Here's the drawing with two shaded views (mm, measured from the low corner). I have some questions. Coordinates: 2 decimals unless noted, no trailing zeros. Write each loop counter-clockwise with the first axis right and the second up, starting at its lowest first coordinate (ties: lowest second). Pieces come first, ordered by that corner, then holes.
Item 1: If we section it at C-C (x = 171.5): Please give me the cut outline in (y, z).
Item 2: If we section it at B-B (z = 68.5): Please give me the cut outline in (x, y).
Item 3: If I drill on line 1 (X direction, y = 1.9, z = 74); line 2 (Z direction, x = 232, y = 1.25); line 3 (Z direction, x = 141, y = 0.3), over which ranges is the centre line in solid material (lowest first)?
Item 4: I'm going to push flat-ended pins straight in: pin 1 Ø1.5 at (x, y) = (19, 2) entering from +Z; pin 2 Ø1.5 at (y, z) = (2, 161.5) entering from +X; pin 3 Ø1.5 at (y, z) = (2, 161.5) entering from -X. Where does each tip first touch, or does it pass through?
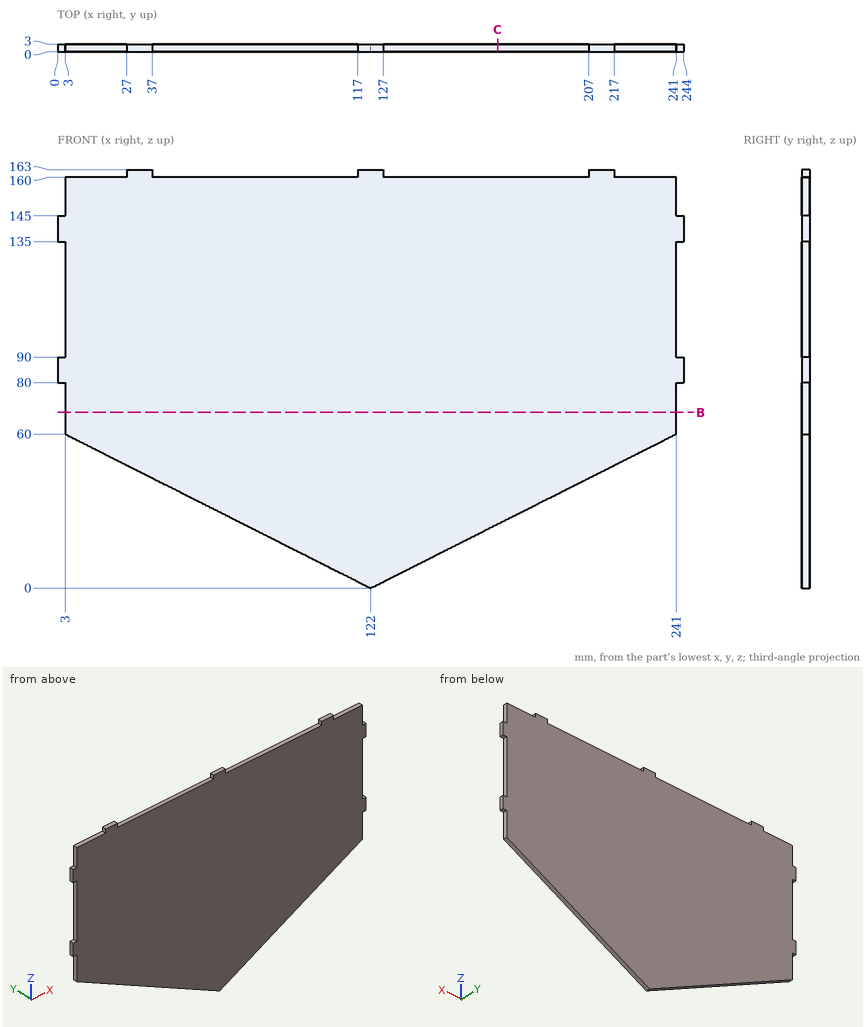
Answer list:
1. outline: (0, 24.96) - (3, 24.96) - (3, 160) - (0, 160) - close
2. outline: (3, 0) - (241, 0) - (241, 3) - (3, 3) - close
3. line 1: x = 3 to 241
3. line 2: z = 55.46 to 160
3. line 3: z = 9.58 to 160
4. pin 1: stops at z = 160
4. pin 2: stops at x = 217
4. pin 3: stops at x = 27
